```python
from build123d import *

# Parameters (mm, degrees)
EXTRUDE_1_DEPTH     = 75
EXTRUDE_START       = 50
EXTRUDE_2_DEPTH     = 4
CHAMFER_1_SIZE      = 2
CUT_EXTRUDE_1_REACH = 237.438
SKETCH_3_W          = 147.5
SKETCH_3_H          = 42
FILLET_1_R          = 3


with BuildPart() as part:
    # 草图1 → 凸台-拉伸1 (new, symmetric)
    with BuildSketch(Plane.XY):
        Polygon((0, 0), (217.5, 0), (217.5, 10), (10, 10), (10, 60), (0, 60), align=None)
    extrude(amount=EXTRUDE_1_DEPTH, both=True)

    # 草图2 → 凸台-拉伸2 (add, symmetric)
    with BuildSketch(Plane.XY.offset(EXTRUDE_START)):
        Polygon((10, 57), (217.5, 20), (217.5, 10), (15, 10), (10, 15), align=None)
    extrude_2 = extrude(amount=EXTRUDE_2_DEPTH, both=True)

    # 倒角1
    chamfer_1_edges = [part.edges().sort_by_distance(p)[0] for p in [
        (217.5, 5, 75),
        (5, 60, 75),
        (5, 60, -75),
        (217.5, 5, -75),
    ]]
    chamfer(chamfer_1_edges, length=CHAMFER_1_SIZE)

    # 镜向1: 凸台-拉伸2 across plane
    add(extrude_2.mirror(Plane.XY))

    # 草图3 → 切除-拉伸1 (cut, up to next)
    with BuildSketch(Plane(origin=(0, 10, 0), x_dir=(1, 0, 0), z_dir=(0, 1, 0)), mode=Mode.PRIVATE) as cut_extrude_1_sk1:
        with Locations((113.75, 0)):
            Rectangle(SKETCH_3_W, SKETCH_3_H)
    cut_extrude_1_tool1 = extrude(cut_extrude_1_sk1.sketch, amount=-CUT_EXTRUDE_1_REACH, mode=Mode.PRIVATE) & part.part
    add(cut_extrude_1_tool1.solids().sort_by_distance((113.75, 10, 0))[0], mode=Mode.SUBTRACT)

    # 圆角1
    fillet_1_edges = [part.edges().sort_by_distance(p)[0] for p in [
        (187.5, 5, -21),
        (187.5, 5, 21),
        (40, 5, 21),
        (40, 5, -21),
    ]]
    fillet(fillet_1_edges, radius=FILLET_1_R)


solid = part.part
```
Work out the finished part from the listing and answer in its coordinate system (mm). A direction names the side the tool comes from. Give positions to 0.01 mm unless a question says otherwise; leave off trailing zeros. Order: outer loops, then holes, each group sorted by start corner. A loop starts at its lowest first (then second) coordinate and runs counter-clockwise, first axis right, second up. Notation, with made-up numbers: (-8.75, 30) - (9.25, 30) arc R8 cw to (9.25, 45) - close; hole circle Ø9 at (-4, 16). An arc over 180 degrees is marked (long way). One line per item, written item: value. Start each with the question number.
1. Consider line 1 (Z direction, x = 119.5, y = 29.5); line 2 (X direction, y = 8, z = 13); line 3 (Z direction, x = 70.5, y = 8). Determine where each line is inside the solid, lowest interval first.
2. Section D-D, the plane y = 31 is taken. Write down the section's boundary in (x, z), then the cut area to 3 significant figures.
3. Section C-C, the plane z = 12.5 is taken. Write down the section's boundary in (x, y).
4. Each of these flat-tipped pins is pushed along its axis until it touches: pin 1 Ø3 at (x, z) = (165.5, -58.5) entering from -Y; pin 2 Ø12 at (x, y) = (98.5, 16.5) entering from +Z; pin 3 Ø8 at (x, y) = (111, 41.5) entering from -Z; pin 4 Ø10 at (x, z) = (166, 58) entering from +Y. Where does it stop, or does it pass through?
5. Which of the six approach directions +Z, -Z, +X, -X, +Y, -Y give full straight-line access (tool end or side, diameter ignored) to faces 4 (the face through (92, 29, -54)), 5 (the face through (92, 29, 46)), 6 (the face through (113, 5, 21)), 7 (the face through (92, 29, 54))?
6. Section B-B, the plane y = 6.5 is taken. Write down the section's boundary in (x, z), then the cut area to 3 significant figures.
7. Section A-A, the plane x = 93 is taken. Write down the section's boundary in (y, z), then the cut area to 3 significant figures.
8. For a pull along Y with two mould halves and no side action, classify faces 1 (the face through (13, 12, 50)), 2 (the face through (5, 60, 1)), 3 (the face through (217.5, 8, 1)) as released by +Y, released by -Y, zero draft, split by the parting line, or undercut.
Filled sheet:
1. line 1: -54 to -46, 46 to 54
1. line 2: 0 to 40, 187.5 to 217.5
1. line 3: -75 to -21, 21 to 75
2. outline: (0, -75) - (10, -75) - (10, -54) - (155.81, -54) - (155.81, -46) - (10, -46) - (10, 46) - (155.81, 46) - (155.81, 54) - (10, 54) - (10, 75) - (0, 75) - close
2. area: 3,830 mm²
3. outline: (0, 0) - (40, 0) - (40, 10) - (10, 10) - (10, 60) - (0, 60) - close; (187.5, 0) - (217.5, 0) - (217.5, 10) - (187.5, 10) - close
4. pin 1: y = 0
4. pin 2: z = 54
4. pin 3: z = -54
4. pin 4: y = 29.72
5. face 4: -Z, +X, +Y
5. face 5: +X, +Y
5. face 6: +Y, -Y
5. face 7: +Z, +X, +Y
6. outline: (0, -75) - (215.5, -75) - (217.5, -73) - (217.5, 73) - (215.5, 75) - (0, 75) - close; hole (40, -18) arc R3 ccw to (43, -21) - (184.5, -21) arc R3 ccw to (187.5, -18) - (187.5, 18) arc R3 ccw to (184.5, 21) - (43, 21) arc R3 ccw to (40, 18) - close
6. area: 26,400 mm²
7. outline: (0, -75) - (10, -75) - (10, -54) - (42.2, -54) - (42.2, -46) - (10, -46) - (10, -21) - (0, -21) - close; (0, 21) - (10, 21) - (10, 46) - (42.2, 46) - (42.2, 54) - (10, 54) - (10, 75) - (0, 75) - close
7. area: 1,600 mm²
8. face 1: undercut
8. face 2: released by +Y
8. face 3: zero draft
